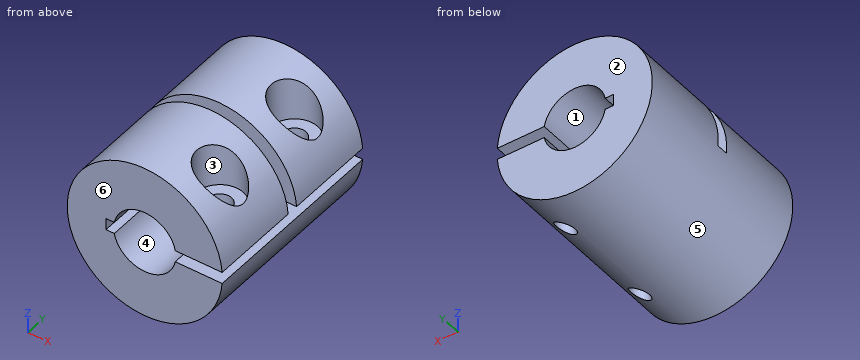
```python
from build123d import *

# Parameters (mm, degrees)
SKETCH2_R               = 10
SKETCH2_R_2             = 4
BOSS_EXTRUDE1_DEPTH     = 25
CUT_EXTRUDE1_DEPTH      = 25
CUT_EXTRUDE1_DEPTH_BACK = 25
SKETCH3_W               = 10.75
SKETCH3_H               = 1.5
SKETCH4_W               = 17.874578158
SKETCH4_H               = 1.5
CUT_EXTRUDE2_DEPTH      = 29.722813233
SKETCH5_R               = 3
CUT_EXTRUDE3_DEPTH      = 6
SKETCH6_R               = 1.5
CUT_EXTRUDE4_DEPTH      = 4
M3_TAPPED_HOLE3_D       = 2.5


with BuildPart() as part:
    # Sketch2 → Boss-Extrude1 (new body)
    with BuildSketch(Plane(origin=(0, 0, 0), x_dir=(1, 0, 0), z_dir=(0, 1, 0))):
        with Locations(Location((0, 0, 0), (0, 0, 270))):
            Circle(SKETCH2_R)
        with Locations(Location((0, 0, 0), (0, 0, 270))):
            Circle(SKETCH2_R_2, mode=Mode.SUBTRACT)
    extrude(amount=BOSS_EXTRUDE1_DEPTH)

    # Sketch3 → Cut-Extrude1 (cut, two sides: drawn at the far end of the back side and taken through both)
    with BuildSketch(Plane(origin=(0, 0, 0), x_dir=(0, 0, -1), z_dir=(1, 0, 0)).offset(-CUT_EXTRUDE1_DEPTH_BACK)):
        with Locations((-4.625, 12.5)):
            Rectangle(SKETCH3_W, SKETCH3_H)
    extrude(amount=CUT_EXTRUDE1_DEPTH + CUT_EXTRUDE1_DEPTH_BACK, mode=Mode.SUBTRACT)

    # Sketch4 → Cut-Extrude2 (cut, through all)
    with BuildSketch(Plane(origin=(0, 25, 0), x_dir=(1, 0, 0), z_dir=(0, 1, 0))):
        with Locations((3.937289079, 0)):
            Rectangle(SKETCH4_W, SKETCH4_H)
    extrude(amount=-CUT_EXTRUDE2_DEPTH, mode=Mode.SUBTRACT)

    # Sketch5 → Cut-Extrude3 (cut)
    with BuildSketch(Plane.XY.offset(10)):
        with Locations((5.429058411, 19.125)):
            Circle(SKETCH5_R)
        with Locations((5.429058411, 5.875)):
            Circle(SKETCH5_R)
    extrude(amount=-CUT_EXTRUDE3_DEPTH, mode=Mode.SUBTRACT)

    # Sketch6 → Cut-Extrude4 (cut)
    with BuildSketch(Plane.XY.offset(4)):
        with Locations((5.429058411, 5.875)):
            Circle(SKETCH6_R)
        with Locations((5.429058411, 19.125)):
            Circle(SKETCH6_R)
    extrude(amount=-CUT_EXTRUDE4_DEPTH, mode=Mode.SUBTRACT)

    # M3 Tapped Hole3 (through all)
    with Locations(Plane.XY.offset(-0.75)):
        with Locations((5.429058411, 19.125), (5.429058411, 5.875)):
            Hole(M3_TAPPED_HOLE3_D / 2)


solid = part.part
```
Geometry check sheet. Reference: the model listing, model coordinates, mm. Face numbers are marked on the shaded views. A direction names the side the tool comes from. Give positions to 0.01 mm unless a question says otherwise; leave off trailing zeros. Order: outer loops, then holes, each group sorted by start corner. A loop starts at its lowest first (then second) coordinate and runs counter-clockwise, first axis right, second up. Notation, with made-up numbers: (42, -30.5) - (57, -30.5) arc R21 ccw to (57, -23.5) - close; hole circle Ø11 at (49, 43). An arc over 180 degrees is marked (long way). Answer in a Markdown table with one row per item. Add a question column.
Q1. Cross-section at D-D, the plane z = -5. Enter the section's corners in (x, y) (3 decimals).
Q2. Gauge pin test, flat ends, axial feed: pin 1 (5 mm diameter, centred on x = 5.43, y = 19.12, fed in from +Z); pin 2 (5 mm diameter, centred on x = -5.5, y = 15, fed in from -Z); pin 3 (3 mm diameter, centred on x = 8.5, y = 4.5, fed in from -Z); pin 4 (2 mm diameter, centred on x = 5.43, y = 5.88, fed in from +Z). Record the tip position at first contact, or that the pin passes through.
Q3. Cross-section at B-B, the plane x = 0. Enter the section's corners in (y, z), then the cut area to 3 significant figures.
Q4. Mould release check, pull along Z, two halves, no side actions. Record for the marked faces 4, 5 and 6: pulls with the +Z half, pulls with the -Z half, needs draft (parallel to the pull), parting line crosses it, or undercut.
Q5. Cross-section at C-C, the plane y = 11. Enter the section's corners in (x, z), then the cut area to 3 significant figures.
Q6. Tool access check on the marked faces 1, 2 and 3. Record the directions out of +Z, -Z, +X, -X, +Y, -Y that give a thin tool (end or side, any length) a straight path to the whole face; none if there is none.
Q7. Material ranges on probe 1 along X at (y, z) = (3.75, 3.25); probe 2 along X at (y, z) = (17, 1); probe 3 along Z at (x, y) = (2.75, 9.25), recorded low to high. Write a range as from..to.
Q8. Cross-section at A-A, the plane z = 0. Enter the section's corners in (x, y).
Check values:
| question | item | result |
|---|---|---|
| 1 | outline | (-8.66, 0) - (8.66, 0) - (8.66, 25) - (-8.66, 25) - close; hole circle Ø2.5 at (5.429, 5.875); hole circle Ø2.5 at (5.429, 19.125) |
| 2 | pin 1 | stops at z = 4 |
| 2 | pin 2 | stops at z = -9.54 |
| 2 | pin 3 | stops at z = -7.14 |
| 2 | pin 4 | passes through |
| 3 | outline | (0, -10) - (25, -10) - (25, -4) - (0, -4) - close; (0, 4) - (11.75, 4) - (11.75, 10) - (0, 10) - close; (13.25, 4) - (25, 4) - (25, 10) - (13.25, 10) - close |
| 3 | area | 291 mm^2 |
| 4 | face 4 | undercut |
| 4 | face 5 | parting line crosses it |
| 4 | face 6 | needs draft |
| 5 | outline | (-5, -0.75) - (-5, 0.75) - (-3.93, 0.75) arc R4 cw to (3.93, 0.75) - (9.97, 0.75) arc R10 ccw (long way) to (9.97, -0.75) - (3.93, -0.75) arc R4 cw to (-3.93, -0.75) - close |
| 5 | area | 253 mm^2 |
| 6 | face 1 | +Y, -Y |
| 6 | face 2 | +Z, -Z, +X, -X, +Y |
| 6 | face 3 | +Z |
| 7 | probe 1 | x = -9.46..-2.33, 2.33..9.46 |
| 7 | probe 2 | x = -9.95..-3.87, 3.87..9.95 |
| 7 | probe 3 | z = -9.61..-2.9, 2.9..9.61 |
| 8 | outline | (-10, 0) - (-5, 0) - (-5, 11.75) - (-10, 11.75) - close; (-10, 13.25) - (-5, 13.25) - (-5, 25) - (-10, 25) - close |
